Design review of the part built by this model. Coordinates are the model's own, in mm. Face numbers are marked on the shaded views. A direction names the side the tool comes from. Round coordinates to 2 decimals unless told otherwise and drop trailing zeros. Loops run counter-clockwise (first coordinate to the right, second up) from the corner with the lowest first, then second, coordinate; pieces in that order, holes last. Notation, with made-up numbers: (-21, 67) -> (-4, 67) arc R13 cw to (-4, 75) -> close; hole circle Ø9 at (39, 70.25). An arc over 180 degrees is marked (long way). Use a Markdown table: item, result. Add a question column.
from build123d import *

# Parameters (mm, degrees)
EXTRUDE_1_DEPTH              = 4
CHAMFER_1_SIZE               = 1
CHAMFER_2_SIZE               = 10
CUT_EXTRUDE_1_REACH          = 56.672
SKETCH_2_R                   = 6.8
HOLE_WIZARD_M4_2_D           = 4.5
HOLE_WIZARD_M4_2_CBORE_D     = 7.5
HOLE_WIZARD_M4_2_CBORE_DEPTH = 4.6
F_4_0MM_1_D                  = 4
F_4_0MM_1_DEPTH              = 10
F_4_0MM_1_TIP                = 1.201721238
HOLE_WIZARD_M4_1_D           = 4.5


with BuildPart() as part:
    # 草图1 → 凸台-拉伸1 (new, symmetric)
    with BuildSketch(Plane(origin=(0, 0, 0), x_dir=(1, 0, 0), z_dir=(0, 1, 0))):
        with BuildLine():
            Line((-30, 0), (30, 0))
            Line((30, 0), (30, 8))
            Line((30, 8), (18, 8))
            ThreePointArc((18, 8), (16.585786438, 8.585786438), (16, 10))
            Line((16, 10), (16, 45))
            Line((16, 45), (-16, 45))
            Line((-16, 45), (-16, 10))
            ThreePointArc((-16, 10), (-16.585786438, 8.585786438), (-18, 8))
            Line((-18, 8), (-30, 8))
            Line((-30, 8), (-30, 0))
        make_face()
    extrude(amount=EXTRUDE_1_DEPTH, both=True)

    # 倒角1
    chamfer_1_edges = [part.edges().sort_by_distance(p)[0] for p in [
        (30, 4, -4),
        (30, -4, -4),
        (-30, -4, -4),
        (-30, 4, -4),
    ]]
    chamfer(chamfer_1_edges, length=CHAMFER_1_SIZE)

    # 倒角2
    chamfer_2_edges = [part.edges().sort_by_distance(p)[0] for p in [
        (-16, 0, -45),
        (16, 0, -45),
    ]]
    chamfer(chamfer_2_edges, length=CHAMFER_2_SIZE)

    # 草图2 → 切除-拉伸1 (cut, up to next)
    with BuildSketch(Plane(origin=(0, 4, 0), x_dir=(1, 0, 0), z_dir=(0, 1, 0)), mode=Mode.PRIVATE) as cut_extrude_1_sk1:
        with Locations(Location((0, 25, 0), (0, 0, 270))):
            Circle(SKETCH_2_R)
    cut_extrude_1_tool1 = extrude(cut_extrude_1_sk1.sketch, amount=-CUT_EXTRUDE_1_REACH, mode=Mode.PRIVATE) & part.part
    add(cut_extrude_1_tool1.solids().sort_by_distance((0, 4, -25))[0], mode=Mode.SUBTRACT)

    # M4 六角圆柱头螺钉的柱形沉头孔2 (through all)
    with Locations(Plane(origin=(0, 4, 0), x_dir=(1, 0, 0), z_dir=(0, 1, 0))):
        with Locations((0, 36), (0, 14)):
            CounterBoreHole(HOLE_WIZARD_M4_2_D / 2, HOLE_WIZARD_M4_2_CBORE_D / 2, HOLE_WIZARD_M4_2_CBORE_DEPTH)

    # Ø4.0mm 暗销孔1
    with Locations(Plane.XY):
        with Locations((-12.5, 0), (12.5, 0)):
            Hole(F_4_0MM_1_D / 2, depth=F_4_0MM_1_DEPTH)
            with Locations((0, 0, -(F_4_0MM_1_DEPTH + F_4_0MM_1_TIP / 2))):  # 118° drill point
                Cone(0, F_4_0MM_1_D / 2, F_4_0MM_1_TIP, mode=Mode.SUBTRACT)

    # M4 间隙孔1 (through all)
    with Locations(Plane(origin=(0, 0, -8), x_dir=(-1, 0, 0), z_dir=(0, 0, -1))):
        with Locations((-25, 0), (25, 0)):
            Hole(HOLE_WIZARD_M4_1_D / 2)


solid = part.part
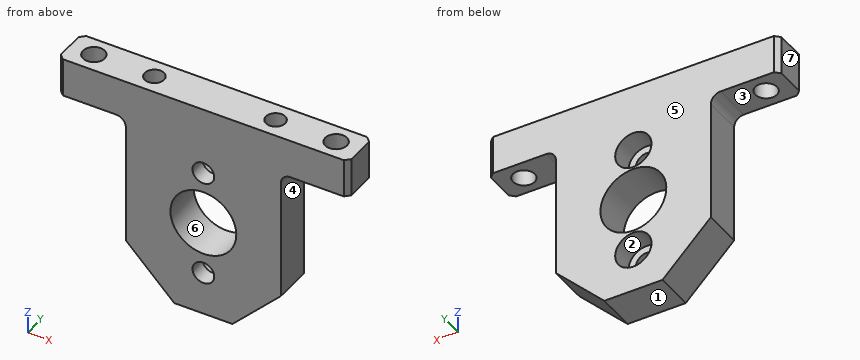
1. Insertion check: P1, Ø4, axis at y = 0.5, z = -30, coming from the -X side; P2, Ø4, axis at y = 1, z = -25.5, coming from the +X side; P3, Ø4, axis at x = 25, y = 0, coming from the +Z side; P4, Ø4, axis at x = 27, y = -1.5, coming from the -Z side. Each pin has a flat end and moves straight along its axis. Give the tip position at first contact, or say it passes through.
2. Consider section A-A on x = 0. State the section outline as (y, z) points, plus the area to 3 significant figures.
3. Consider section B-B on z = -7. State the section outline as (x, y) points.
4. To check wall thickness, follow probe 1 along X at (y, z) = (1.5, -25); probe 2 along Y at (x, z) = (-12.5, -2.25); probe 3 along X at (y, z) = (1, -1.5). State the ranges of each line that lie inside material, in increasing order. Write a range as from..to.
5. Consider section C-C on x = -25. State the section outline as (y, z) points.
6. Mouldability with a two-part tool opening along X and no side actions: class the marked faces 5, 6 and 7 as +X half, -X half, draft (parallel to the pull), parting line (faces both ways), or undercut.
7. Consider section D-D on z = -14. State the section outline as (x, y) points.
8. For the marked faces 1, 2, 3 and 4, list the 3-axis set-ups (+Z, -Z, +X, -X, +Y, -Y) from which the entire face can be reached by the end or side of a thin tool; tool diameter is ignored.
Verdict:
| question | item | result |
|---|---|---|
| 1 | P1 | stops at x = -16 |
| 1 | P2 | stops at x = 16 |
| 1 | P3 | passes through |
| 1 | P4 | stops at z = -8 |
| 2 | outline | (-4, -45) -> (4, -45) -> (4, -39.75) -> (-0.6, -39.75) -> (-0.6, -38.25) -> (-4, -38.25) -> close; (-4, -33.75) -> (-0.6, -33.75) -> (-0.6, -32.25) -> (4, -32.25) -> (4, -31.8) -> (-4, -31.8) -> close; (-4, -18.2) -> (4, -18.2) -> (4, -17.75) -> (-0.6, -17.75) -> (-0.6, -16.25) -> (-4, -16.25) -> close; (-4, -11.75) -> (-0.6, -11.75) -> (-0.6, -10.25) -> (4, -10.25) -> (4, 0) -> (-4, 0) -> close |
| 2 | area | 152 mm² |
| 3 | outline | (-30, -3) -> (-29, -4) -> (29, -4) -> (30, -3) -> (30, 3) -> (29, 4) -> (-29, 4) -> (-30, 3) -> close; hole circle Ø4.5 at (-25, 0); hole circle Ø4 at (-12.5, 0); hole circle Ø4 at (12.5, 0); hole circle Ø4.5 at (25, 0) |
| 4 | probe 1 | x = -16..-6.8, 6.8..16 |
| 4 | probe 2 | y = -4..-2, 2..4 |
| 4 | probe 3 | x = -30..-27.02, -22.98..-14.23, -10.77..10.77, 14.23..22.98, 27.02..30 |
| 5 | outline | (-4, -8) -> (-2.25, -8) -> (-2.25, 0) -> (-4, 0) -> close; (2.25, -8) -> (4, -8) -> (4, 0) -> (2.25, 0) -> close |
| 6 | face 5 | draft |
| 6 | face 6 | undercut |
| 6 | face 7 | -X half |
| 7 | outline | (-16, -4) -> (-2.25, -4) -> (-2.25, -0.6) -> (-3.75, -0.6) -> (-3.75, 4) -> (-16, 4) -> close; (2.25, -4) -> (16, -4) -> (16, 4) -> (3.75, 4) -> (3.75, -0.6) -> (2.25, -0.6) -> close |
| 8 | face 1 | -Z, +X, -X, +Y, -Y |
| 8 | face 2 | +Y |
| 8 | face 3 | -Z, -X, +Y, -Y |
| 8 | face 4 | -Z, +X, +Y, -Y |
